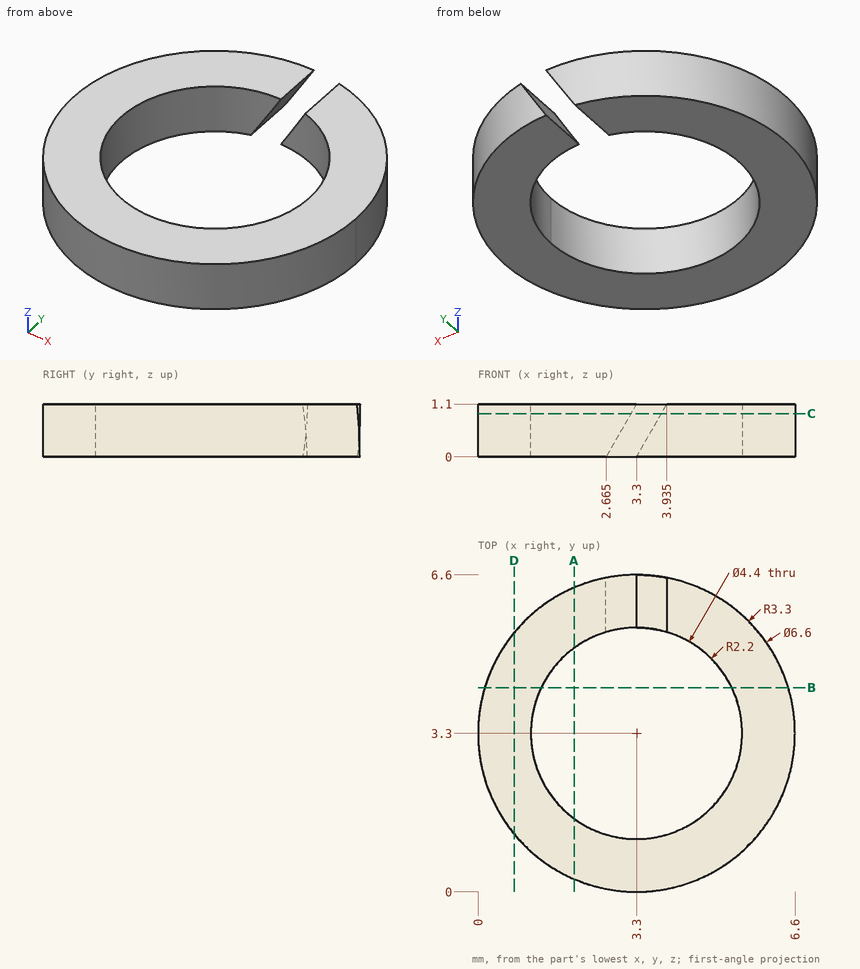
Check sheet for the drawn part. Datum: minimum x, y, z corner. Units: mm. Give positions to 0.01 mm unless a question says otherwise; leave off trailing zeros. Order: outer loops, then holes, each group sorted by start corner. A loop starts at its lowest first (then second) coordinate and runs counter-clockwise, first axis right, second up.
1. Sectioned sample at C-C (z = 0.9). Record the boundary of the cut face in (x, y).
Completed:
outline: (3.18, 5.5) - (3.18, 6.6) arc R3.3 ccw (long way) to (3.82, 6.56) - (3.82, 5.44) arc R2.2 cw (long way) to start
2. Scan lines: line 1 (X direction, y = 3.3, z = 0.85); line 2 (Y direction, x = 3.3, z = 0.75); line 3 (Y direction, x = 2.5, z = 0.9). Record each from-to range of solid material in increasing order.
Completed:
line 1: x = 0 to 1.1, 5.5 to 6.6
line 2: y = 0 to 1.1
line 3: y = 0.1 to 1.25, 5.35 to 6.5
3. Sectioned sample at B-B (y = 4.25). Record the boundary of the cut face in (x, z), then the cut area to 3 significant figures.
Completed:
outline: (0.14, 0) - (1.32, 0) - (1.32, 1.1) - (0.14, 1.1) - close; (5.28, 0) - (6.46, 0) - (6.46, 1.1) - (5.28, 1.1) - close
area: 2.59 mm2
4. Sectioned sample at A-A (x = 2). Record the boundary of the cut face in (y, z) (3 decimals), then the cut area to 3 significant figures.
Completed:
outline: (0.267, 0) - (1.525, 0) - (1.525, 1.1) - (0.267, 1.1) - close; (5.075, 0) - (6.333, 0) - (6.333, 1.1) - (5.075, 1.1) - close
area: 2.77 mm2
5. Depth check by flat-ended pin: pin 1 (3 mm diameter, centred on x = 2, y = 4, fed in from +Z). Enter the tip coordinate at first touch or a pass-through.
Completed:
pin 1: stops at z = 1.1
6. Sectioned sample at D-D (x = 0.75). Record the boundary of the cut face in (y, z), then the cut area to 3 significant figures.
Completed:
outline: (1.21, 0) - (5.39, 0) - (5.39, 1.1) - (1.21, 1.1) - close
area: 4.61 mm2
